Part model, mm, in its own coordinate system. Give positions to 0.01 mm unless a question says otherwise; leave off trailing zeros. Order: outer loops, then holes, each group sorted by start corner. A loop starts at its lowest first (then second) coordinate and runs counter-clockwise, first axis right, second up. Notation, with made-up numbers: M 23,25 L 39,25 A30 cw 39,61 Z; hole C 37,34 d7. An arc over 180 degrees is marked long. One line per question, with ' | ' between items.
```python
from build123d import *

# Parameters (mm, degrees)
SKETCH_1_W         = 34
SKETCH_1_H         = 8
EXTRUDE_1_DEPTH    = 8
HOLE_WIZARD_M3_1_D = 2.5
HOLE_WIZARD_M3_2_D = 2.5


with BuildPart() as part:
    # 草图1 → 凸台-拉伸1 (new body)
    with BuildSketch(Plane(origin=(0, 0, 0), x_dir=(1, 0, 0), z_dir=(0, 1, 0))):
        Rectangle(SKETCH_1_W, SKETCH_1_H)
    extrude(amount=EXTRUDE_1_DEPTH)

    # M3 螺纹孔1 (through all)
    with Locations(Plane(origin=(0, 8, 0), x_dir=(1, 0, 0), z_dir=(0, 1, 0))):
        with Locations((4, 0), (-12, 0)):
            Hole(HOLE_WIZARD_M3_1_D / 2)

    # M3 螺纹孔2 (through all)
    with Locations(Plane.XY.offset(4)):
        with Locations((12, 4), (-4, 4)):
            Hole(HOLE_WIZARD_M3_2_D / 2)


solid = part.part
```
1. Slice it at B-B on x = 4. Give the cut face in (y, z), then the cut area to 3 significant figures.
Worked out:
outline: M 0,-4 L 8,-4 L 8,-1.25 L 0,-1.25 Z; M 0,1.25 L 8,1.25 L 8,4 L 0,4 Z | area: 44.0 mm2
2. Slice it at C-C on y = 7.25. Give the cut face in (x, z).
Worked out:
outline: M -17,-4 L 17,-4 L 17,4 L -17,4 Z; hole C -12,0 d2.5; hole C 4,0 d2.5
3. Mould opens along X. For faces 1 (the flat face through (0, 8, 0)), 2 (the cylindrical face through (-10.75, 3.94, -0.05)), 3 (the flat face through (17, 4, 0)), 4 (the flat face through (-17, 4, 0)) say: released by +X, released by -X, zero draft, split by the parting line, or undercut.
Worked out:
face 1: zero draft | face 2: undercut | face 3: released by +X | face 4: released by -X
4. Slice it at A-A on z = 0. Give the cut face in (x, y), then the cut area to 3 significant figures.
Worked out:
outline: M -17,0 L -13.25,0 L -13.25,8 L -17,8 Z; M -10.75,0 L 2.75,0 L 2.75,8 L -10.75,8 Z; M 5.25,0 L 17,0 L 17,8 L 5.25,8 Z; hole C -4,4 d2.5; hole C 12,4 d2.5 | area: 222 mm2
5. Slice it at D-D on z = 3.5. Give the cut face in (x, y), then the cut area to 3 significant figures.
Worked out:
outline: M -17,0 L 17,0 L 17,8 L -17,8 Z; hole C -4,4 d2.5; hole C 12,4 d2.5 | area: 262 mm2
6. Probe L1, parallel to Z at x = 4, y = 3.75; L2, parallel to Y at x = 12, z = -2; L3, parallel to X at y = 5, z = 2.75. List the from-to ranges inside material, lowest first. Write a range as from..to.
Worked out:
L1: z = -4..-1.25, 1.25..4 | L2: y = 0..2.75, 5.25..8 | L3: x = -17..-4.75, -3.25..11.25, 12.75..17
